Geometry check sheet. Reference: drawing and pictorial views, mm from the part's lowest x, y, z. A direction names the side the tool comes from. Coordinates: 2 decimals unless noted, no trailing zeros. Order: outer loops, then holes, each group sorted by start corner. A loop starts at its lowest first (then second) coordinate and runs counter-clockwise, first axis right, second up. Notation, with made-up numbers: (-24.75, 86) -> (29.25, 86) arc R23 cw to (29.25, 100) -> close; hole circle Ø1 at (38, 46.5). An arc over 180 degrees is marked (long way). Use CSV: the item, a comma, the result in double quotes. Start each with the question number.
1) Sectioned sample at B-B on x = 90. Record the boundary of the cut face in (y, z).
2) Scan lines: line 1 along Z through (x, y) = (10, 31.2); line 2 along X through (y, z) = (12, 26); line 3 along X through (y, z) = (33, 7). Record each from-to range of solid material in increasing order.
3) Go/stop test with flat-tipped pins: pin 1 (4 mm diameter, centred on x = 83, z = 11, fed in from -Y); pin 2 (3.5 mm diameter, centred on x = 10, z = 7.5, fed in from +Y); pin 3 (5 mm diameter, centred on x = 60.5, z = 8.5, fed in from +Y); pin 4 (9 mm diameter, centred on y = 21, z = 16.5, fed in from +X). Record where each tip stops, or that it passes through.
4) Tool access check on the marked faces 1, 2, 3 and 4. Record the directions out of +Z, -Z, +X, -X, +Y, -Y that give a thin tool (end or side, any length) a straight path to the whole face; none if there is none.
5) Sectioned sample at D-D on z = 14. Record the boundary of the cut face in (x, y).
6) Sectioned sample at A-A on z = 7.5. Record the boundary of the cut face in (x, y), then the cut area to 3 significant figures.
7) Sectioned sample at C-C on y = 7.5. Record the boundary of the cut face in (x, z).
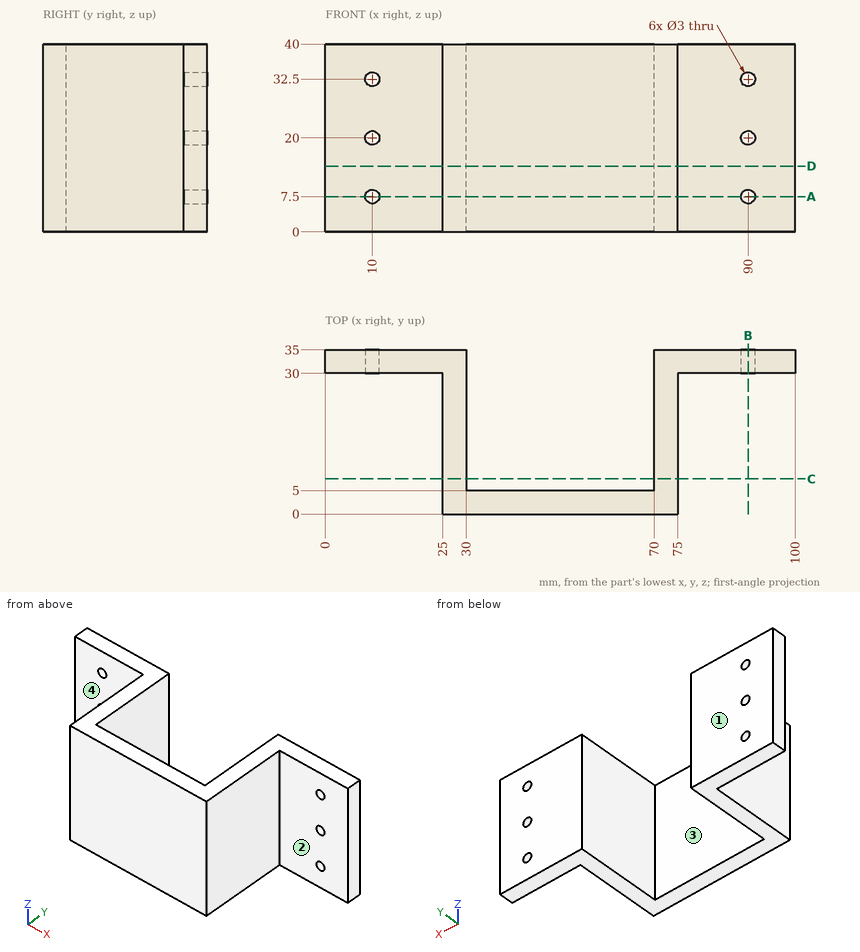
Answers follow:
1,outline,"(30, 0) -> (35, 0) -> (35, 6) -> (30, 6) -> close; (30, 9) -> (35, 9) -> (35, 18.5) -> (30, 18.5) -> close; (30, 21.5) -> (35, 21.5) -> (35, 31) -> (30, 31) -> close; (30, 34) -> (35, 34) -> (35, 40) -> (30, 40) -> close"
2,line 1,"z = 0 to 6, 9 to 18.5, 21.5 to 31, 34 to 40"
2,line 2,"x = 25 to 30, 70 to 75"
2,line 3,"x = 0 to 8.59, 11.41 to 30, 70 to 88.59, 91.41 to 100"
3,pin 1,"stops at y = 30"
3,pin 2,"stops at y = 35"
3,pin 3,"stops at y = 5"
3,pin 4,"stops at x = 75"
4,face 1,"+Z, -Z, +X, -X, +Y"
4,face 2,"+Z, -Z, +X, -Y"
4,face 3,"+Z, -Z, +Y"
4,face 4,"+Z, -Z, -X, -Y"
5,outline,"(0, 30) -> (25, 30) -> (25, 0) -> (75, 0) -> (75, 30) -> (100, 30) -> (100, 35) -> (70, 35) -> (70, 5) -> (30, 5) -> (30, 35) -> (0, 35) -> close"
6,outline,"(0, 30) -> (8.5, 30) -> (8.5, 35) -> (0, 35) -> close; (11.5, 30) -> (25, 30) -> (25, 0) -> (75, 0) -> (75, 30) -> (88.5, 30) -> (88.5, 35) -> (70, 35) -> (70, 5) -> (30, 5) -> (30, 35) -> (11.5, 35) -> close; (91.5, 30) -> (100, 30) -> (100, 35) -> (91.5, 35) -> close"
6,area,"770 mm²"
7,outline,"(25, 0) -> (30, 0) -> (30, 40) -> (25, 40) -> close; (70, 0) -> (75, 0) -> (75, 40) -> (70, 40) -> close"
